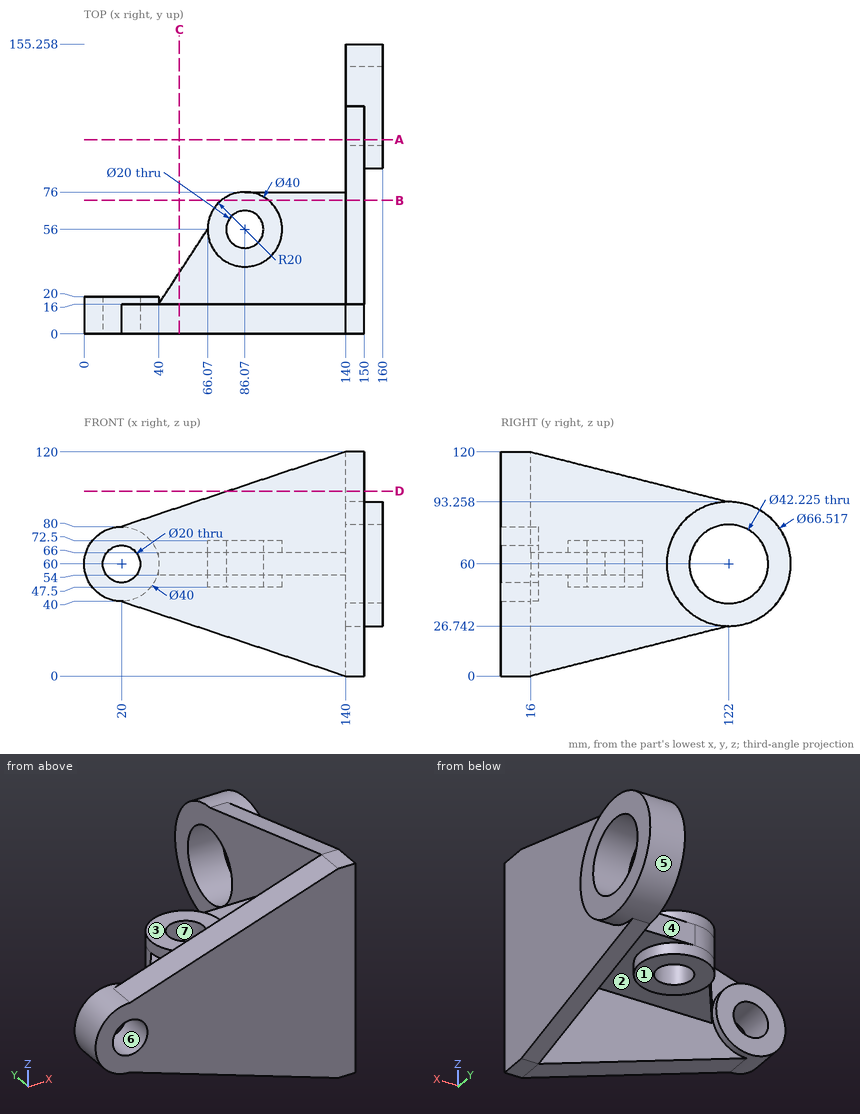
Input: dimensioned drawing with shaded views. Units: mm. Origin: part minimum x, y, z. A direction names the side the tool comes from. Give positions to 0.01 mm unless a question says otherwise; leave off trailing zeros. Loops run counter-clockwise (first coordinate to the right, second up) from the corner with the lowest first, then second, coordinate; pieces in that order, holes last. Notation, with made-up numbers: (33, 4) -> (46, 4) arc R34 cw to (46, 38) -> close; hole circle Ø1 at (10.25, 50). An arc over 180 degrees is marked (long way). Use a Markdown table: item, result. Add a question column.
1) Section query C-C, the plane x = 51. Return the cut outline in (y, z), then the cut area to 3 significant figures.
2) Reachability of the marked faces 1, 2, 3 and 4 from +Z, -Z, +X, -X, +Y, -Y: full face, straight path, thin tool, end or side. Return the list, or none.
3) First-contact query: pin 1 (9.5 mm diameter, centred on x = 121, z = 57.5, fed in from +Y); pin 2 (6 mm diameter, centred on y = 79.5, z = 90.5, fed in from +X); pin 3 (23 mm diameter, centred on x = 86.07, y = 56, fed in from +Z). Flat tips, straight axial feed; report the tip coordinate or a pass-through.
4) Section query A-A, the plane y = 104. Return the cut outline in (x, z), then the cut area to 3 significant figures.
5) Line query: line 1 along Y through (x, z) = (86.07, 54.25); line 2 along X through (y, z) = (15.25, 60); line 3 along Y through (x, z) = (108, 29). Output: solid intervals per line, ascending. Write a range as [from, to].
6) Section query D-D, the plane z = 99. Return the cut outline in (x, y).
7) Section query B-B, the plane y = 71.5. Return the cut outline in (x, z).
8) Pull-direction query (Z, two-part tool) for the marked faces 5, 6 and 7; classes: +Z half, -Z half, draft (parallel to the pull), parting line (faces both ways), or undercut.
Numbers:
| question | item | result |
|---|---|---|
| 1 | outline | (0, 29.67) -> (16, 29.67) -> (16, 54) -> (32.88, 54) -> (32.88, 66) -> (16, 66) -> (16, 90.33) -> (0, 90.33) -> close |
| 1 | area | 1,170 mm2 |
| 2 | face 1 | -Z, -X, +Y |
| 2 | face 2 | -Z |
| 2 | face 3 | +Z, -X, +Y |
| 2 | face 4 | +Z, -Z, -X, +Y |
| 3 | pin 1 | stops at y = 76 |
| 3 | pin 2 | stops at x = 150 |
| 3 | pin 3 | stops at z = 72.5 |
| 4 | outline | (140, 22.2) -> (150, 22.2) -> (150, 32.03) -> (160, 32.03) -> (160, 48.97) -> (140, 48.97) -> close; (140, 71.03) -> (160, 71.03) -> (160, 87.97) -> (150, 87.97) -> (150, 97.8) -> (140, 97.8) -> close |
| 4 | area | 874 mm2 |
| 5 | line 1 | y = [0, 46], [66, 76] |
| 5 | line 2 | x = [0, 10], [30, 150] |
| 5 | line 3 | y = [0, 16] |
| 6 | outline | (77, 0) -> (150, 0) -> (150, 99.24) -> (140, 99.24) -> (140, 16) -> (77, 16) -> close |
| 7 | outline | (73.43, 47.5) -> (98.71, 47.5) -> (98.71, 54) -> (140, 54) -> (140, 14) -> (150, 14) -> (150, 106) -> (140, 106) -> (140, 66) -> (98.71, 66) -> (98.71, 72.5) -> (73.43, 72.5) -> close |
| 8 | face 5 | parting line |
| 8 | face 6 | undercut |
| 8 | face 7 | draft |
